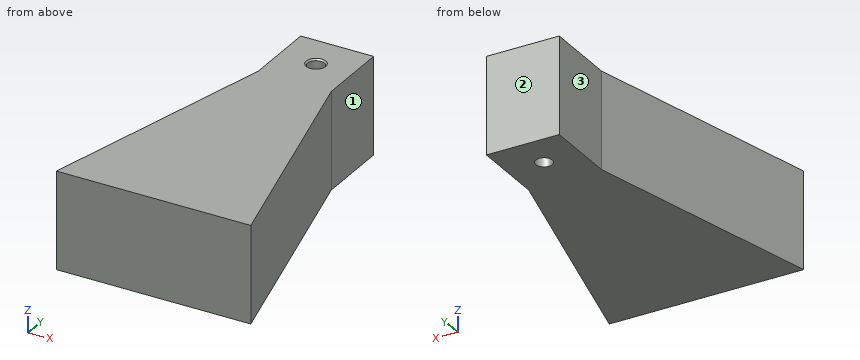
from build123d import *

# Parameters (mm, degrees)
BOSS_EXTRUDE1_DEPTH         = 40
M8_TAPPED_HOLE1_D           = 6.8
M8_TAPPED_HOLE1_CSINK_D     = 8.05
M8_TAPPED_HOLE1_CSINK_ANGLE = 90


with BuildPart() as part:
    # Sketch1 → Boss-Extrude1 (new body)
    with BuildSketch(Plane.XY):
        Polygon((40, -72.727272727), (-40, -72.727272727), (-15, 27.272727273), (-15, 57.272727273), (15, 57.272727273), (15, 27.272727273), align=None)
    extrude(amount=BOSS_EXTRUDE1_DEPTH)

    # M8 Tapped Hole1 (through all)
    with Locations(Plane.XY.offset(40)):
        with Locations((0, 42.272727273)):
            CounterSinkHole(M8_TAPPED_HOLE1_D / 2, M8_TAPPED_HOLE1_CSINK_D / 2, counter_sink_angle=M8_TAPPED_HOLE1_CSINK_ANGLE)


solid = part.part
Work out the finished part from the listing and answer in its coordinate system (mm). Face numbers are marked on the shaded views. A direction names the side the tool comes from. Give positions to 0.01 mm unless a question says otherwise; leave off trailing zeros. Order: outer loops, then holes, each group sorted by start corner. A loop starts at its lowest first (then second) coordinate and runs counter-clockwise, first axis right, second up. Notation, with made-up numbers: (70.5, 89) - (116.5, 89) arc R23 cw to (116.5, 98) - close; hole circle Ø8 at (20, -19). An arc over 180 degrees is marked (long way). Answer as CSV lines item,"result". Start each with the question number.
Q1. For the marked faces 1, 2 and 3, determine the directions among +Z, -Z, +X, -X, +Y, -Y from which every point of the face is accessible in a straight line to the end or side of a thin tool.
Q2. Find the intervals of material crossed by L1, parallel to Y at x = 0, z = 9; L2, parallel to X at y = 41.5, z = 10; L3, parallel to X at y = 28.5, z = 4, in increasing order. Write a range as [from, to].
Q3. The part is cut by section C-C (y = -0.5). Write down the section's boundary in (x, z).
Q4. The part is cut by section B-B (z = 29). Write down the section's boundary in (x, y).
Q5. The part is cut by section D-D (x = 28). Write down the section's boundary in (y, z), then the cut area to 3 significant figures.
Q6. Given pin 1 Ø10 at (y, z) = (5, 10.5) entering from +X; pin 2 Ø8 at (y, z) = (34.5, 25) entering from -X; pin 3 Ø1.5 at (y, z) = (-34, 13.5) entering from -X, each flat-ended and moving along its own axis, determine where each tip first touches the part or whether it passes through.
Q7. The part is cut by section A-A (x = 0). Write down the section's boundary in (y, z) (3 decimals).
Check result:
1,face 1,"+Z, -Z, +X, +Y"
1,face 2,"+Z, -Z, +X, -X, +Y"
1,face 3,"+Z, -Z, -X, +Y"
2,L1,"y = [-72.73, 38.87], [45.67, 57.27]"
2,L2,"x = [-15, -3.31], [3.31, 15]"
2,L3,"x = [-15, 15]"
3,outline,"(-21.94, 0) - (21.94, 0) - (21.94, 40) - (-21.94, 40) - close"
4,outline,"(-40, -72.73) - (40, -72.73) - (15, 27.27) - (15, 57.27) - (-15, 57.27) - (-15, 27.27) - close; hole circle Ø6.8 at (0, 42.27)"
5,outline,"(-72.73, 0) - (-24.73, 0) - (-24.73, 40) - (-72.73, 40) - close"
5,area,"1,920 mm²"
6,pin 1,"stops at x = 21.82"
6,pin 2,"stops at x = -15"
6,pin 3,"stops at x = -30.51"
7,outline,"(-72.727, 0) - (38.873, 0) - (38.873, 39.375) - (38.248, 40) - (-72.727, 40) - close; (45.673, 0) - (57.273, 0) - (57.273, 40) - (46.298, 40) - (45.673, 39.375) - close"
